from build123d import *

# Parameters (mm, degrees)
SKETCH1_R      = 8
EXTRUDE1_DEPTH = 9
FILLET1_R      = 1.5


with BuildPart() as part:
    # Sketch1 → Extrude1 (new body)
    with BuildSketch(Plane(origin=(0, 0, 0), x_dir=(1, 0, 0), z_dir=(0, 1, 0))):
        Polygon((13.856406461, 0), (6.92820323, 12), (-6.92820323, 12), (-13.856406461, 0), (-6.92820323, -12), (6.92820323, -12), align=None)
        with Locations(Location((0, 0, 0), (0, 0, 270))):
            Circle(SKETCH1_R, mode=Mode.SUBTRACT)
    extrude(amount=EXTRUDE1_DEPTH)

    # Fillet1
    fillet1_edges = [part.edges().sort_by_distance(p)[0] for p in [
        (0, 0, 12),
        (-10.392304845, 0, 6),
        (-10.392304845, 0, -6),
        (0, 0, -12),
        (10.392304845, 0, -6),
        (10.392304845, 0, 6),
    ]]
    fillet(fillet1_edges, radius=FILLET1_R)


solid = part.part
Verification items for the finished model (mm, model axes). Coordinates: 2 decimals unless noted, no trailing zeros. Loops run counter-clockwise (first coordinate to the right, second up) from the corner with the lowest first, then second, coordinate; pieces in that order, holes last. Notation, with made-up numbers: M 66,9.25 L 104,9.25 A17 cw 104,19.25 Z; hole C 10,68.5 d9. An arc over 180 degrees is marked long. One line per item, written item: value.
1. Section check C-C on y = 1. Record the cut outline in (x, z).
Answers follow:
outline: M -13.76,0 L -6.88,-11.91 L 6.88,-11.91 L 13.76,0 L 6.88,11.91 L -6.88,11.91 Z; hole C 0,0 d16
2. Gauge pin test, flat ends, axial feed: P1, Ø1, axis at x = -8.5, z = 7, coming from the -Y side; P2, Ø1.5, axis at y = 1.5, z = -3.5, coming from the -X side; P3, Ø1, axis at y = 1, z = 8.5, coming from the +X side; P4, Ø5, axis at x = -10.5, y = 5.5, coming from the +Z side. Record the tip position at first contact, or that the pin passes through.
Answers follow:
P1: y = 0
P2: x = -12.27
P3: x = 9.18
P4: z = 10.14
3. Section check A-A on y = 6.75. Record the cut outline in (x, z), plus the area to 3 significant figures.
Answers follow:
outline: M -13.86,0 L -6.93,-12 L 6.93,-12 L 13.86,0 L 6.93,12 L -6.93,12 Z; hole C 0,0 d16
area: 298 mm^2
4. Mould release check, pull along Z, two halves, no side actions. Record for faces 1 (the cylindrical face through (-7.81, 4.44, -1.73)), 2 (the flat face through (8, 0, 2)), 3 (the cylindrical face through (10.07, 0.45, 5.7)): pulls with the +Z half, pulls with the -Z half, needs draft (parallel to the pull), parting line crosses it, or undercut.
Answers follow:
face 1: undercut
face 2: needs draft
face 3: pulls with the +Z half
5. Material ranges on line 1 along Z through (x, y) = (-5, 7.75) (3 decimals); line 2 along Z through (x, y) = (-6.5, 5); line 3 along X through (y, z) = (1.25, -4), recorded low to high. Write a range as from..to.
Answers follow:
line 1: -12..-6.245, 6.245..12
line 2: -12..-4.66, 4.66..12
line 3: -11.52..-6.93, 6.93..11.52
6. Section check B-B on x = 0. Record the cut outline in (y, z).
Answers follow:
outline: M 0,-10.5 A1.5 ccw 1.5,-12 L 9,-12 L 9,-8 L 0,-8 Z; M 0,8 L 9,8 L 9,12 L 1.5,12 A1.5 ccw 0,10.5 Z
